Read the model definition and answer for the solid it produces. Units are mm, in the model's axes. Coordinates: 2 decimals unless noted, no trailing zeros. Write each loop counter-clockwise with the first axis right and the second up, starting at its lowest first coordinate (ties: lowest second). Pieces come first, ordered by that corner, then holes. Notation, with made-up numbers: (63.5, 11.5) -> (87.5, 11.5) arc R20 ccw to (87.5, 15.5) -> close; hole circle Ø4 at (22.25, -38.75). An arc over 180 degrees is marked (long way). Write item = value, one per line. Start each with the question number.
1) Section A-A (z = 1.25) is taken. Determine the outline of the cut face in (x, y).
2) Flat-ended cylindrical pins translate along their axes: pin 1 Ø8 at (x, y) = (-199.5, 132.5) entering from -Z; pin 2 Ø1.5 at (x, y) = (-203.5, 117) entering from -Z; pin 3 Ø3 at (y, z) = (124.5, 1.5) entering from +X. Find the tip coordinate at first contact, or state that the pin passes through.
3) Find the intervals of material crossed by line 1 along X through (y, z) = (26, 2); line 2 along Y through (x, z) = (-211, -2); line 3 along Y through (x, z) = (-174.5, -1.75), in increasing order. Write a range as from..to.
from build123d import *

# Parameters (mm, degrees)
SWEEP1_PROFILE_R   = 3
CUT_EXTRUDE1_DEPTH = 25


with BuildPart() as part:
    # Sweep1: sweep along a path in Sketch1
    with BuildLine(Plane.XY) as sweep1_path:
        ThreePointArc((-173.152744336, 155.907431282), (-217.524239374, 83.499732244), (-233, 0))
    # Sweep1 profile (on start of the path) → Sweep1 (sweep)
    with BuildSketch(Plane(origin=(-173.152744336, 155.907431282, 0), x_dir=(-0.7431448254773938, 0.6691306063588589, 0), z_dir=(-0.6691306063588589, -0.7431448254773938, 0))):
        Circle(SWEEP1_PROFILE_R)
    sweep(path=sweep1_path.line)

    # Sketch6 → Cut-Extrude1 (cut, symmetric)
    with BuildSketch(Plane.XY):
        with BuildLine():
            Line((0, 0), (-230.569138435, 14.102212633))
            ThreePointArc((-230.569138435, 14.102212633), (-230.892259483, 7.054396551), (-231, 0))
            Line((-231, 0), (0, 0))
        make_face()
        with BuildLine():
            Line((0, 0), (-171.666454685, 154.569170069))
            ThreePointArc((-171.666454685, 154.569170069), (-174.997511393, 150.787502819), (-178.245278763, 146.934068884))
            Line((-178.245278763, 146.934068884), (0, 0))
        make_face()
    extrude(amount=CUT_EXTRUDE1_DEPTH, both=True, mode=Mode.SUBTRACT)


solid = part.part
Answer key:
q1.outline = (-235.73, 0) -> (-231, 0) arc R231 cw to (-230.57, 14.1) -> (-229.84, 14.06) arc R230.27 cw to (-177.68, 146.47) -> (-178.25, 146.93) arc R231 cw to (-171.67, 154.57) -> (-175.18, 157.73) arc R235.73 ccw to start
q2.pin_1 = -1.67
q2.pin_2 = -2.83
q2.pin_3 = -192.66
q3.line_1 = -233.79..-229.29
q3.line_2 = 93.44..104
q3.line_3 = 151.36..157.12
